The model under review builds one solid part; all positions refer to its coordinate system, in mm. Round coordinates to 2 decimals unless told otherwise and drop trailing zeros. Loops run counter-clockwise (first coordinate to the right, second up) from the corner with the lowest first, then second, coordinate; pieces in that order, holes last. Notation, with made-up numbers: (14.25, 67.25) -> (52.25, 67.25) arc R24 ccw to (52.25, 81.25) -> close; hole circle Ø11 at (-25, -14.5). An arc over 180 degrees is marked (long way). Return JSON: item names as keys, results as strings. Group by question number.
```python
from build123d import *

# Parameters (mm, degrees)
EXTRUDE_1_DEPTH = 30


with BuildPart() as part:
    # 草图1 → 凸台-拉伸1 (new body)
    with BuildSketch(Plane(origin=(0, 0, 0), x_dir=(1, 0, 0), z_dir=(0, 1, 0))):
        Polygon((0, 0), (0, -228), (-20, -248), (-155.862358683, -248), (-155.862358683, -218), (-30, 0), align=None)
    extrude(amount=EXTRUDE_1_DEPTH)


solid = part.part
```
1. For P1, Ø3, axis at y = 24, z = 213.5, coming from the -X side; P2, Ø10, axis at x = -94, z = 195.5, coming from the -Y side; P3, Ø8, axis at x = -91, y = 9, coming from the -Z side; P4, Ø6, axis at y = 4.5, z = 58, coming from the -X side, all flat-tipped, find the tip position at first contact; note any pin that passes through.
2. We need section B-B, the plane x = -117. Write out the cut boundary in (y, z), then the cut area to 3 significant figures.
3. We need section A-A, the plane y = 14. Write out the cut boundary in (x, z), then the cut area to 3 significant figures.
4. We need section C-C, the plane z = 162.5. Write out the cut boundary in (x, y), then the cut area to 3 significant figures.
5. Wall thickness on line 1 (X direction, y = 6.25, z = 43.5); line 2 (Z direction, x = -62, y = 22); line 3 (X direction, y = 8.5, z = 157.5): over which ranges is each line inside the solid? List them lowest first.
Check sheet entries:
{
 "1": {"P1": "stops at x = -154.13", "P2": "stops at y = 0", "P3": "stops at z = 98.73", "P4": "stops at x = -65.22"},
 "2": {"outline": "(0, 150.69) -> (30, 150.69) -> (30, 248) -> (0, 248) -> close", "area": "2,920 mm²"},
 "3": {"outline": "(-155.86, 218) -> (-30, 0) -> (0, 0) -> (0, 228) -> (-20, 248) -> (-155.86, 248) -> close", "area": "24,700 mm²"},
 "4": {"outline": "(-123.82, 0) -> (0, 0) -> (0, 30) -> (-123.82, 30) -> close", "area": "3,710 mm²"},
 "5": {"line 1": "x = -55.11 to 0", "line 2": "z = 55.43 to 248", "line 3": "x = -120.93 to 0"}
}
